Read the model definition and answer for the solid it produces. Units are mm, in the model's axes. Face numbers are marked on the shaded views. Coordinates: 2 decimals unless noted, no trailing zeros. Order: outer loops, then holes, each group sorted by start corner. A loop starts at its lowest first (then second) coordinate and runs counter-clockwise, first axis right, second up. Notation, with made-up numbers: M 49,-13 L 104,-13 A18 ccw 104,19 Z; hole C 33.5,48 d11. An arc over 180 degrees is marked long. Use a Markdown table: item, result. Add a question column.
1) The mould has two halves that part along X. Classify the marked faces 1, 2, 3 and 4: released by +X, released by -X, zero draft, split by the parting line, or undercut.
2) This flat-tipped pin is pushed along its axis until it touches: pin 1 Ø5 at (x, z) = (-2.5, -1) entering from -Y. Where does it stop, or does it pass through?
3) Find section C-C on x = 3.5. Write down the section's boundary in (y, z).
4) Find section A-A on z = 0. Write down the section's boundary in (x, y), plus the area to 3 significant figures.
5) Find section B-B on y = 1.35. Write down the section's boundary in (x, z).
6) Find section D-D on z = 4.25. Write down the section's boundary in (x, y), plus the area to 3 significant figures.
7) Find the intervals of material crossed by probe 1 along X at (y, z) = (1.4, 2.25); probe 2 along X at (y, z) = (1.7, 1.75); probe 3 along Z at (x, y) = (-0.25, 1.4), in increasing order. Write a range as [from, to].
from build123d import *

# Parameters (mm, degrees)
EXTRUDE_1_DEPTH    = 2.4
HOLE_WIZARD_M6_1_D = 5


with BuildPart() as part:
    # 草图1 → 凸台-拉伸1 (new body)
    with BuildSketch(Plane(origin=(0, 0, 0), x_dir=(1, 0, 0), z_dir=(0, 1, 0))):
        Polygon((0, 5.773502692), (-5, 2.886751346), (-5, -2.886751346), (0, -5.773502692), (5, -2.886751346), (5, 2.886751346), align=None)
    extrude(amount=EXTRUDE_1_DEPTH)

    # M6 螺纹孔1 (through all)
    with Locations(Plane(origin=(0, 2.4, 0), x_dir=(1, 0, 0), z_dir=(0, 1, 0))):
        with Locations((0, 0)):
            Hole(HOLE_WIZARD_M6_1_D / 2)


solid = part.part
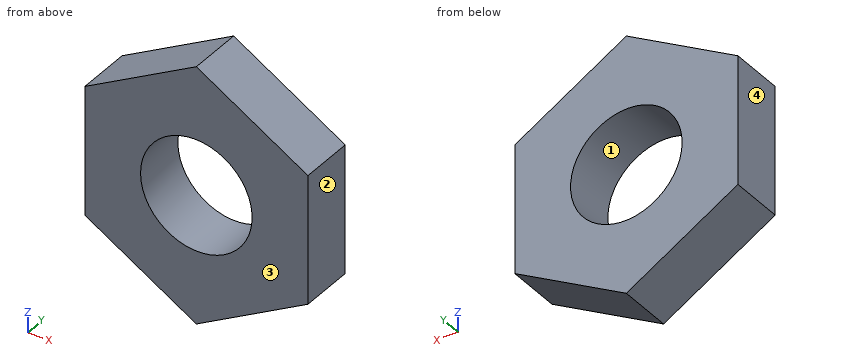
Check result:
| question | item | result |
|---|---|---|
| 1 | face 1 | undercut |
| 1 | face 2 | released by +X |
| 1 | face 3 | zero draft |
| 1 | face 4 | released by -X |
| 2 | pin 1 | stops at y = 0 |
| 3 | outline | M 0,-3.75 L 2.4,-3.75 L 2.4,3.75 L 0,3.75 Z |
| 4 | outline | M -5,0 L -2.5,0 L -2.5,2.4 L -5,2.4 Z; M 2.5,0 L 5,0 L 5,2.4 L 2.5,2.4 Z |
| 4 | area | 12.0 mm2 |
| 5 | outline | M -5,-2.89 L 0,-5.77 L 5,-2.89 L 5,2.89 L 0,5.77 L -5,2.89 Z; hole C 0,0 d5 |
| 6 | outline | M -2.64,0 L 2.64,0 L 2.64,2.4 L -2.64,2.4 Z |
| 6 | area | 12.7 mm2 |
| 7 | probe 1 | x = [-5, -1.09], [1.09, 5] |
| 7 | probe 2 | x = [-5, -1.79], [1.79, 5] |
| 7 | probe 3 | z = [-5.63, -2.49], [2.49, 5.63] |
